from build123d import *

# Parameters (mm, degrees)
SKETCH1_W          = 110
SKETCH1_H          = 4
SKETCH2_W          = 4
SKETCH2_H          = 2
CUT_EXTRUDE1_DEPTH = 5
CHAMFER1_SIZE      = 0.5


with BuildPart() as part:
    # Sketch1 → Revolve1 (revolve)
    with BuildSketch(Plane.XY, mode=Mode.PRIVATE) as revolve1_sk:
        with Locations((55, 2)):
            Rectangle(SKETCH1_W, SKETCH1_H)
    revolve(revolve1_sk.sketch.rotate(Axis((0, 0, 0), (1, 0, 0)), 90), axis=Axis((0, 0, 0), (1, 0, 0)))

    # Sketch2 → Cut-Extrude1 (cut, symmetric)
    with BuildSketch(Plane(origin=(0, 0, 0), x_dir=(1, 0, 0), z_dir=(0, 1, 0))):
        with Locations((4, 4)):
            Rectangle(SKETCH2_W, SKETCH2_H)
    extrude(amount=CUT_EXTRUDE1_DEPTH, both=True, mode=Mode.SUBTRACT)

    # Chamfer1
    chamfer1_edges = [part.edges().sort_by_distance(p)[0] for p in [
        (110, 0, -4),
        (0, 0, -4),
    ]]
    chamfer(chamfer1_edges, length=CHAMFER1_SIZE)


solid = part.part
For this review, take the finished solid that the model builds, in its own axes (mm). Round coordinates to 2 decimals unless told otherwise and drop trailing zeros. Order: outer loops, then holes, each group sorted by start corner. A loop starts at its lowest first (then second) coordinate and runs counter-clockwise, first axis right, second up. Notation, with made-up numbers: (54, -17) -> (58, -17) arc R22 ccw to (58, -8) -> close; hole circle Ø8 at (30.5, -15.5). An arc over 180 degrees is marked (long way). Put each result on its own line as item: value.
Q1. Add section A-A on x = 99.5. Write out the cut boundary in (y, z).
Check result:
outline: circle Ø8 at (0, 0)
Q2. Mouldability with a two-part tool opening along X and no side actions: class faces 1 (the flat face through (0, 0, 0)), 2 (the flat face through (110, 0, 0)), 3 (the flat face through (4, 0, -3)) as pulls with the +X half, pulls with the -X half, needs draft (parallel to the pull), parting line crosses it, or undercut.
Check result:
face 1: pulls with the -X half
face 2: pulls with the +X half
face 3: undercut
Q3. Insertion check: pin 1 Ø1.2 at (x, y) = (5, -1) entering from -Z. The pin has a flat end and moves straight along its axis. Give the tip position at first contact, or say it passes through.
Check result:
pin 1: z = -3
Q4. For probe 1 along Z at (x, y) = (55, -0.25); probe 2 along Z at (x, y) = (62, -3); probe 3 along X at (y, z) = (-1, -3.5), list the stretches that pass through material, from the lowest coordinate up. Write a range as [from, to].
Check result:
probe 1: [-3.99, 3.99]
probe 2: [-2.65, 2.65]
probe 3: [0.14, 2], [6, 109.86]
